from build123d import *

# Parameters (mm, degrees)
SKETCH_1_W          = 10
SKETCH_1_H          = 20
EXTRUDE_1_DEPTH     = 7
SKETCH_2_W          = 4
SKETCH_2_H          = 4
SKETCH_2_R          = 1.1
EXTRUDE_2_DEPTH     = 7
FILLET_1_R          = 1
SKETCH_3_W          = 5.954377652
SKETCH_3_H          = 2.653951182
CUT_EXTRUDE_1_DEPTH = 0.1


with BuildPart() as part:
    # 草图1 → 凸台-拉伸1 (new body)
    with BuildSketch(Plane.XY):
        Rectangle(SKETCH_1_W, SKETCH_1_H)
    extrude(amount=EXTRUDE_1_DEPTH)

    # 草图2 → 凸台-拉伸2 (add)
    # profile 1 of 2: a face of its own
    with BuildSketch(Plane.XY.offset(7)):
        with Locations((7, 4.5)):
            Rectangle(SKETCH_2_W, SKETCH_2_H)
        with Locations((7, 4.5)):
            Circle(SKETCH_2_R, mode=Mode.SUBTRACT)
    # profile 2 of 2: a face of its own
    with BuildSketch(Plane.XY.offset(7)):
        with Locations((7, -4.5)):
            Rectangle(SKETCH_2_W, SKETCH_2_H)
        with Locations((7, -4.5)):
            Circle(SKETCH_2_R, mode=Mode.SUBTRACT)
    extrude(amount=-EXTRUDE_2_DEPTH)

    # 圆角1
    fillet_1_edges = [part.edges().sort_by_distance(p)[0] for p in [
        (5, -10, 3.5),
        (-5, -10, 3.5),
        (5, 10, 3.5),
        (-5, 10, 3.5),
    ]]
    fillet(fillet_1_edges, radius=FILLET_1_R)

    # 草图3 → 切除-拉伸1 (cut)
    with BuildSketch(Plane.ZY.offset(5)):
        with Locations((3.551037523, 7.111228168)):
            Rectangle(SKETCH_3_W, SKETCH_3_H)
    cut_extrude_1 = extrude(amount=-CUT_EXTRUDE_1_DEPTH, mode=Mode.SUBTRACT)

    # 镜向1: 切除-拉伸1 across plane
    add(cut_extrude_1.mirror(Plane.ZX), mode=Mode.SUBTRACT)


solid = part.part
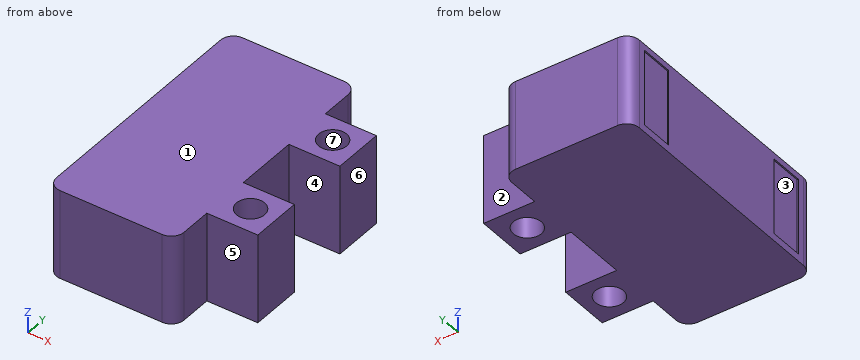
Here's how the part is built. I have some questions about the finished solid (model axes, mm). Face numbers are marked on the shaded views. A direction names the side the tool comes from. Give positions to 0.01 mm unless a question says otherwise; leave off trailing zeros. Loops run counter-clockwise (first coordinate to the right, second up) from the corner with the lowest first, then second, coordinate; pieces in that order, holes last. Notation, with made-up numbers: (74, 66.25) -> (90, 66.25) arc R31 ccw to (90, 101.25) -> close; hole circle Ø8 at (-11.75, -16.75). An arc over 180 degrees is marked (long way). Answer as a JSON object with one key per item and string values. Group by question number.
Item 1: Will these pins go through, and if not, where does the flat tip stop? pin 1 (3 mm diameter, centred on x = 7.5, z = 5, fed in from -Y); pin 2 (2 mm diameter, centred on x = 7.5, z = 2.5, fed in from +Y); pin 3 (1.3 mm diameter, centred on y = -7, z = 3, fed in from -X).
Item 2: Thinking about a two-plate mould opening in X: for the marked faces 5, 6 and 7, which applies, pulls with the +X half, pulls with the -X half, needs draft (parallel to the pull), parting line crosses it, or undercut?
Item 3: Imagine slicing it at B-B on z = 2.25. Write out the boundary of the cut face in (x, y).
Item 4: On a 3-axis mill with a long thin cutter (end or side, diameter ignored), from which of +Z, -Z, +X, -X, +Y, -Y can I reach the whole of each face in a straight line? I mean the marked faces 1, 2, 3 and 4. Say none if no direction works.
Item 5: Imagine slicing it at C-C on x = 7. Write out the boundary of the cut face in (y, z).
Item 6: Imagine slicing it at A-A on y = -4.5. Write out the boundary of the cut face in (x, z).
Item 7: I need wall thicknesses on L1, parallel to Y at x = 7, z = 5.25; L2, parallel to Y at x = 6, z = 4; L3, parallel to X at y = -4, z = 4.75. Which ranges of each line are inside material? Lowest first, please.
Item 8: Imagine slicing it at D-D on x = 5.25. Write out the boundary of the cut face in (y, z), then the cut area to 3 significant figures.
Answer list:
{
 "1": {"pin 1": "stops at y = -6.5", "pin 2": "stops at y = 6.5", "pin 3": "stops at x = -4.9"},
 "2": {"face 5": "needs draft", "face 6": "pulls with the +X half", "face 7": "undercut"},
 "3": {"outline": "(-5, -9) arc R1 ccw to (-4, -10) -> (4, -10) arc R1 ccw to (5, -9) -> (5, -6.5) -> (9, -6.5) -> (9, -2.5) -> (5, -2.5) -> (5, 2.5) -> (9, 2.5) -> (9, 6.5) -> (5, 6.5) -> (5, 9) arc R1 ccw to (4, 10) -> (-4, 10) arc R1 ccw to (-5, 9) -> (-5, 8.44) -> (-4.9, 8.44) -> (-4.9, 5.78) -> (-5, 5.78) -> (-5, -5.78) -> (-4.9, -5.78) -> (-4.9, -8.44) -> (-5, -8.44) -> close; hole circle Ø2.2 at (7, -4.5); hole circle Ø2.2 at (7, 4.5)"},
 "4": {"face 1": "+Z, +X, -X, +Y, -Y", "face 2": "+Z, -Z, +X, +Y", "face 3": "-X", "face 4": "+Z, -Z, +X"},
 "5": {"outline": "(-6.5, 0) -> (-5.6, 0) -> (-5.6, 7) -> (-6.5, 7) -> close; (-3.4, 0) -> (-2.5, 0) -> (-2.5, 7) -> (-3.4, 7) -> close; (2.5, 0) -> (3.4, 0) -> (3.4, 7) -> (2.5, 7) -> close; (5.6, 0) -> (6.5, 0) -> (6.5, 7) -> (5.6, 7) -> close"},
 "6": {"outline": "(-5, 0) -> (5.9, 0) -> (5.9, 7) -> (-5, 7) -> close; (8.1, 0) -> (9, 0) -> (9, 7) -> (8.1, 7) -> close"},
 "7": {"L1": "y = -6.5 to -5.6, -3.4 to -2.5, 2.5 to 3.4, 5.6 to 6.5", "L2": "y = -6.5 to -4.96, -4.04 to -2.5, 2.5 to 4.04, 4.96 to 6.5", "L3": "x = -5 to 6.02, 7.98 to 9"},
 "8": {"outline": "(-6.5, 0) -> (-2.5, 0) -> (-2.5, 7) -> (-6.5, 7) -> close; (2.5, 0) -> (6.5, 0) -> (6.5, 7) -> (2.5, 7) -> close", "area": "56.0 mm2"}
}
